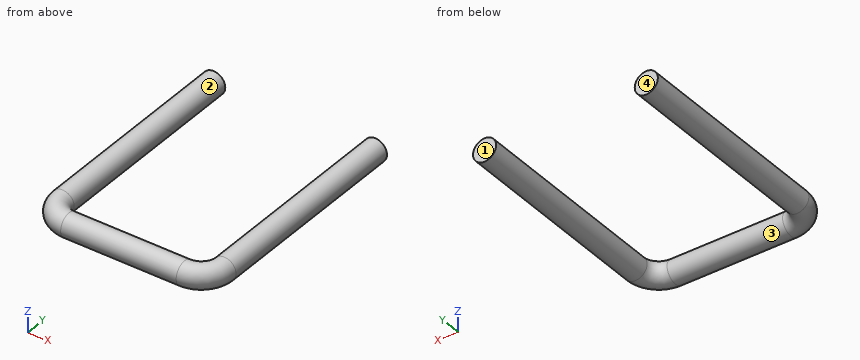
```python
from build123d import *

# Parameters (mm, degrees)
SWEEP1_PROFILE_R = 5


with BuildPart() as part:
    # Sweep1: sweep along a path in Sketch1
    with BuildLine(Plane.XY) as sweep1_path:
        Line((-35, 100), (-35, 10))
        ThreePointArc((-35, 10), (-32.071067812, 2.928932188), (-25, 0))
        Line((-25, 0), (25, 0))
        ThreePointArc((25, 0), (32.071067812, 2.928932188), (35, 10))
        Line((35, 10), (35, 100))
    # Sweep1 profile (on start of the path) → Sweep1 (sweep)
    with BuildSketch(Plane(origin=(-35, 100, 0), x_dir=(0, 0, -1), z_dir=(0, -1, 0))):
        Circle(SWEEP1_PROFILE_R)
    sweep(path=sweep1_path.line)


solid = part.part
```
The listing builds one solid part. Answer for the finished solid, in the listing's coordinates (mm). Face numbers are marked on the shaded views. A direction names the side the tool comes from. Give positions to 0.01 mm unless a question says otherwise; leave off trailing zeros. Write each loop counter-clockwise with the first axis right and the second up, starting at its lowest first coordinate (ties: lowest second). Pieces come first, ordered by that corner, then holes. Notation, with made-up numbers: (28, 59) - (77, 59) arc R18 cw to (77, 89) - close; hole circle Ø2 at (76, 83.5). An arc over 180 degrees is marked (long way). Use one line per item in the form item = value. Start each with the question number.
1) Find section C-C on x = 1.5. Determine the outline of the cut face in (y, z), plus the area to 3 significant figures.
2) Find section B-B on y = 51.5. Determine the outline of the cut face in (x, z), plus the area to 3 significant figures.
3) Consider line 1 along X through (y, z) = (94, 0.5); line 2 along X through (y, z) = (50.5, 3.5); line 3 along Y through (x, z) = (13.5, 0.5). Determine where each line is inside the solid, lowest interval first. Write a range as from..to.
4) A tool of negligible diameter and unlimited length cuts with its end or side. For the marked faces 1 and 2, from which of +Z, -Z, +X, -X, +Y, -Y can it reach the whole face along a straight path? Write none if from no direction.
5) The mould has two halves that part along X. Classify the marked faces 3 and 4: pulls with the +X half, pulls with the -X half, needs draft (parallel to the pull), parting line crosses it, or undercut.
6) Flat-ended cylindrical pins translate along their axes: pin 1 Ø5 at (x, z) = (15, 0.5) entering from +Y; pin 2 Ø5 at (x, z) = (29.5, 2.5) entering from -Y; pin 3 Ø5 at (y, z) = (83, 3.5) entering from -X. Find the tip coordinate at first contact, or state that the pin passes through.
7) Find section A-A on z = 0. Determine the outline of the cut face in (x, y).
Geometry results:
q1.outline = circle Ø10 at (0, 0)
q1.area = 78.5 mm2
q2.outline = circle Ø10 at (-35, 0); circle Ø10 at (35, 0)
q2.area = 157 mm2
q3.line_1 = -39.97..-30.03, 30.03..39.97
q3.line_2 = -38.57..-31.43, 31.43..38.57
q3.line_3 = -4.97..4.97
q4.face_1 = +Z, -Z, +X, -X, +Y
q4.face_2 = +Y
q5.face_3 = undercut
q5.face_4 = needs draft
q6.pin_1 = 5
q6.pin_2 = -4.7
q6.pin_3 = -39.9
q7.outline = (-40, 10) arc R15 ccw to (-25, -5) - (25, -5) arc R15 ccw to (40, 10) - (40, 100) - (30, 100) - (30, 10) arc R5 cw to (25, 5) - (-25, 5) arc R5 cw to (-30, 10) - (-30, 100) - (-40, 100) - close
